Geometry: see drawing. Coordinates: mm, zero at the bounding-box minimum. Coordinates: 2 decimals unless noted, no trailing zeros. Order: outer loops, then holes, each group sorted by start corner. A loop starts at its lowest first (then second) coordinate and runs counter-clockwise, first axis right, second up.
Item 1: Section B-B on z = 7.15. Return the cut outline in (x, y), then the cut area to 4 significant figures.
Item 2: Ray query, line 1 (Z direction, x = 19, y = 1.6); line 2 (Z direction, x = 22, y = 2.05); line 3 (X direction, y = 1.35, z = 41). Return the intervals inside material, ascending.
Item 3: Section C-C on x = 12. Return the cut outline in (y, z).
Item 4: Contact query for a flat-ended pin moving along its axis: P1, Ø6.5, axis at x = 27.5, z = 8, coming from the +Y side. Output: stop coordinate, or through.
Item 5: Section A-A on x = 20.5. Return the cut outline in (y, z).
Item 6: Section D-D on z = 40. Return the cut outline in (x, y), then the cut area to 3 significant figures.
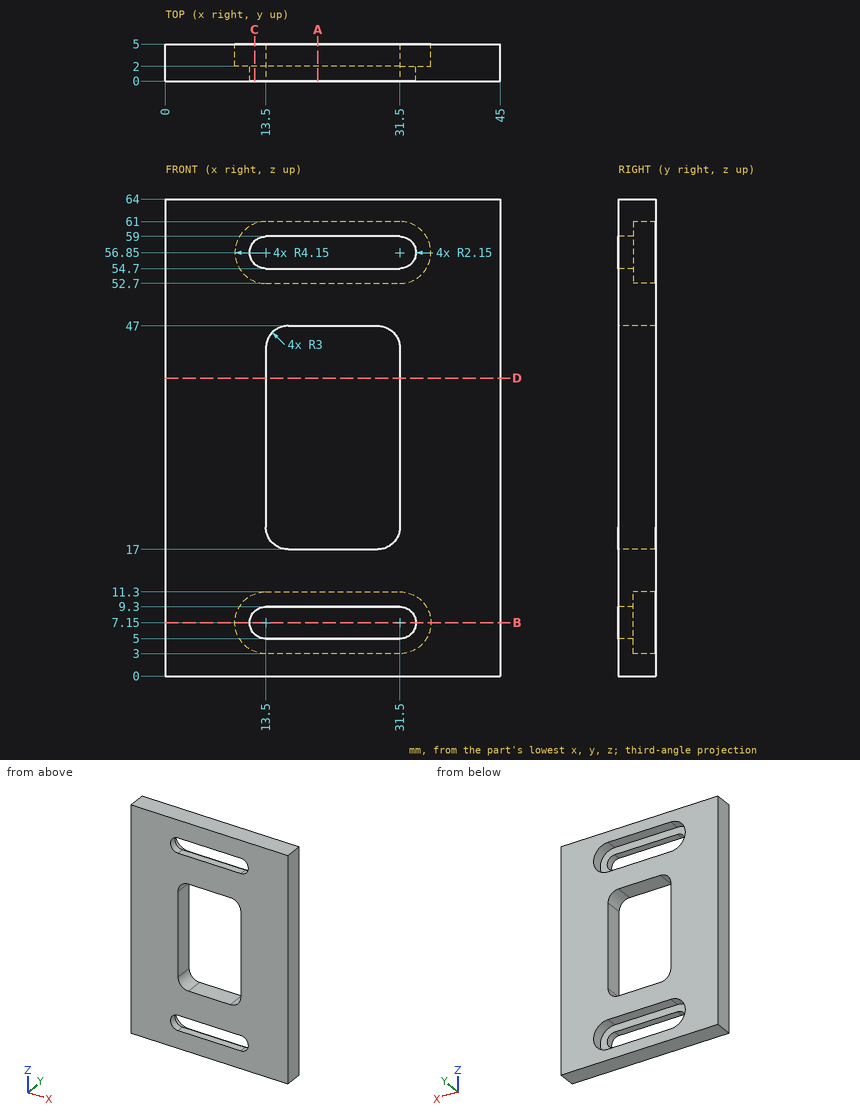
Answer list:
1. outline: (0, 0) - (11.35, 0) - (11.35, 2) - (9.35, 2) - (9.35, 5) - (0, 5) - close; (33.65, 0) - (45, 0) - (45, 5) - (35.65, 5) - (35.65, 2) - (33.65, 2) - close
1. area: 101.5 mm2
2. line 1: z = 0 to 5, 9.3 to 17, 47 to 54.7, 59 to 64
2. line 2: z = 0 to 3, 11.3 to 17, 47 to 52.7, 61 to 64
2. line 3: x = 0 to 13.5, 31.5 to 45
3. outline: (0, 0) - (5, 0) - (5, 3.28) - (2, 3.28) - (2, 5.61) - (0, 5.61) - close; (0, 8.69) - (2, 8.69) - (2, 11.02) - (5, 11.02) - (5, 52.98) - (2, 52.98) - (2, 55.31) - (0, 55.31) - close; (0, 58.39) - (2, 58.39) - (2, 60.72) - (5, 60.72) - (5, 64) - (0, 64) - close
4. P1: stops at y = 2
5. outline: (0, 0) - (5, 0) - (5, 3) - (2, 3) - (2, 5) - (0, 5) - close; (0, 9.3) - (2, 9.3) - (2, 11.3) - (5, 11.3) - (5, 17) - (0, 17) - close; (0, 47) - (5, 47) - (5, 52.7) - (2, 52.7) - (2, 54.7) - (0, 54.7) - close; (0, 59) - (2, 59) - (2, 61) - (5, 61) - (5, 64) - (0, 64) - close
6. outline: (0, 0) - (13.5, 0) - (13.5, 5) - (0, 5) - close; (31.5, 0) - (45, 0) - (45, 5) - (31.5, 5) - close
6. area: 135 mm2
